```python
from build123d import *

# Parameters (mm, degrees)
SKETCH1_W                      = 75
SKETCH1_H                      = 165
BOSS_EXTRUDE1_DEPTH            = 80
SHELL1_T                       = -6
FILLET1_R                      = 6
FILLET2_R                      = 3
CHAMFER1_SIZE                  = 2
M4_TAPPED_HOLE1_D              = 3.3
F_6_5_6_5_DIAMETER_HOLE1_D     = 6.5
F_6_5_6_5_DIAMETER_HOLE1_DEPTH = 10
F_6_5_6_5_DIAMETER_HOLE1_TIP   = 1.952797012
M5_TAPPED_HOLE1_D              = 4.2


with BuildPart() as part:
    # Sketch1 → Boss-Extrude1 (new body)
    with BuildSketch(Plane.XY):
        Rectangle(SKETCH1_W, SKETCH1_H)
    extrude(amount=BOSS_EXTRUDE1_DEPTH)

    # Shell1
    shell1_openings = [part.faces().sort_by_distance(p)[0] for p in [
        (0, 0, 0),
        (0, -82.5, 40),
        (-37.5, 0, 40),
        (37.5, 0, 40),
    ]]
    offset(amount=SHELL1_T, openings=shell1_openings, kind=Kind.INTERSECTION)

    # Fillet1
    fillet1_edges = [part.edges().sort_by_distance(p)[0] for p in [
        (0, 82.5, 80),
    ]]
    fillet(fillet1_edges, radius=FILLET1_R)

    # Fillet2
    fillet2_edges = [part.edges().sort_by_distance(p)[0] for p in [
        (0, 76.5, 74),
    ]]
    fillet(fillet2_edges, radius=FILLET2_R)

    # Chamfer1
    chamfer1_edges = [part.edges().sort_by_distance(p)[0] for p in [
        (-37.5, 79.5, 0),
        (37.5, 79.5, 0),
        (37.5, -82.5, 77),
        (-37.5, -82.5, 77),
    ]]
    chamfer(chamfer1_edges, length=CHAMFER1_SIZE)

    # M4 Tapped Hole1 (through all)
    with Locations(Plane(origin=(0, 0, 74), x_dir=(-1, 0, 0), z_dir=(0, 0, -1))):
        with Locations((-12.5, -72.5), (-12.5, 11.5), (12.5, 11.5), (12.5, -72.5)):
            Hole(M4_TAPPED_HOLE1_D / 2)

    # Ø6.5 (6.5) Diameter Hole1
    with Locations(Plane.XZ.offset(-76.5)):
        with Locations((-20, 10), (20, 10)):
            Hole(F_6_5_6_5_DIAMETER_HOLE1_D / 2, depth=F_6_5_6_5_DIAMETER_HOLE1_DEPTH)
            with Locations((0, 0, -(F_6_5_6_5_DIAMETER_HOLE1_DEPTH + F_6_5_6_5_DIAMETER_HOLE1_TIP / 2))):  # 118° drill point
                Cone(0, F_6_5_6_5_DIAMETER_HOLE1_D / 2, F_6_5_6_5_DIAMETER_HOLE1_TIP, mode=Mode.SUBTRACT)

    # M5 Tapped Hole1 (through all)
    with Locations(Plane(origin=(0, 0, 74), x_dir=(-1, 0, 0), z_dir=(0, 0, -1))):
        with Locations((-17.5, 34.5), (17.5, 34.5)):
            Hole(M5_TAPPED_HOLE1_D / 2)


solid = part.part
```
Verification items for the finished model (mm, model axes). A direction names the side the tool comes from. Coordinates: 2 decimals unless noted, no trailing zeros. Loops run counter-clockwise (first coordinate to the right, second up) from the corner with the lowest first, then second, coordinate; pieces in that order, holes last. Notation, with made-up numbers: (76.5, 61.25) -> (84.5, 61.25) arc R13 ccw to (84.5, 66.25) -> close; hole circle Ø9 at (47.5, 9). An arc over 180 degrees is marked (long way). Answer in a Markdown table with one row per item.
1) Section check D-D (x = 6). Record the cut outline in (y, z).
The answers:
| item | result |
|---|---|
| outline | (-82.5, 74) -> (73.5, 74) arc R3 cw to (76.5, 71) -> (76.5, 0) -> (82.5, 0) -> (82.5, 74) arc R6 ccw to (76.5, 80) -> (-82.5, 80) -> close |
2) Scan lines: line 1 along X through (y, z) = (11, 77); line 2 along X through (y, z) = (34, 77); line 3 along Z through (x, y) = (-4, -12). Record each from-to range of solid material in increasing order. Write a range as from..to.
The answers:
| item | result |
|---|---|
| line 1 | x = -37.5..-14.07, -10.93..10.93, 14.07..37.5 |
| line 2 | x = -37.5..-19.54, -15.46..15.46, 19.54..37.5 |
| line 3 | z = 74..80 |
3) Section check C-C (y = 11.5). Record the cut outline in (x, z), and give its area (3 significant figures).
The answers:
| item | result |
|---|---|
| outline | (-37.5, 74) -> (-14.15, 74) -> (-14.15, 80) -> (-37.5, 80) -> close; (-10.85, 74) -> (10.85, 74) -> (10.85, 80) -> (-10.85, 80) -> close; (14.15, 74) -> (37.5, 74) -> (37.5, 80) -> (14.15, 80) -> close |
| area | 410 mm2 |
4) Depth check by flat-ended pin: P1, Ø5, axis at x = -20.5, z = 51.5, coming from the -Y side; P2, Ø2, axis at x = 12.5, y = -72.5, coming from the +Z side; P3, Ø4.5, axis at x = -12.5, y = -72.5, coming from the -Z side. Enter the tip coordinate at first touch or a pass-through.
The answers:
| item | result |
|---|---|
| P1 | stops at y = 76.5 |
| P2 | passes through |
| P3 | stops at z = 74 |
5) Section check B-B (z = 10). Record the cut outline in (x, y).
The answers:
| item | result |
|---|---|
| outline | (-37.5, 76.5) -> (-23.25, 76.5) -> (-23.25, 82.5) -> (-37.5, 82.5) -> close; (-16.75, 76.5) -> (16.75, 76.5) -> (16.75, 82.5) -> (-16.75, 82.5) -> close; (23.25, 76.5) -> (37.5, 76.5) -> (37.5, 82.5) -> (23.25, 82.5) -> close |
6) Draft check along X on faces 1 (the face through (0.52, 75.6, 73.14)), 2 (the face through (-37.5, 25, 75)), 3 (the face through (-16.531, 32.637, 77.042)). Enter one of: released by +X, released by -X, zero draft, split by the parting line, or undercut.
The answers:
| item | result |
|---|---|
| face 1 | zero draft |
| face 2 | released by -X |
| face 3 | undercut |
7) Access from +Z, -Z, +X, -X, +Y, -Y to the whole of each face (thin tool, end or side, straight path). Record for faces 4 (the face through (-1, 76.5, 35)), 5 (the face through (0, -82.5, 77)).
The answers:
| item | result |
|---|---|
| face 4 | -Z, +X, -X, -Y |
| face 5 | +Z, -Z, +X, -X, -Y |
8) Section check A-A (x = -12.5). Record the cut outline in (y, z).
The answers:
| item | result |
|---|---|
| outline | (-82.5, 74) -> (-74.15, 74) -> (-74.15, 80) -> (-82.5, 80) -> close; (-70.85, 74) -> (9.85, 74) -> (9.85, 80) -> (-70.85, 80) -> close; (13.15, 74) -> (73.5, 74) arc R3 cw to (76.5, 71) -> (76.5, 0) -> (82.5, 0) -> (82.5, 74) arc R6 ccw to (76.5, 80) -> (13.15, 80) -> close |
